Check sheet for the modelled part. Datum: model origin and axes. Units: mm. A direction names the side the tool comes from. Round coordinates to 2 decimals unless told otherwise and drop trailing zeros. Write each loop counter-clockwise with the first axis right and the second up, starting at its lowest first coordinate (ties: lowest second). Pieces come first, ordered by that corner, then holes. Notation, with made-up numbers: M 8,-17 L 54,-17 A20 cw 54,22 Z; hole C 31.5,35.25 d11. An arc over 180 degrees is marked long. Put each result on its own line as item: value.
```python
from build123d import *

# Parameters (mm, degrees)
SKETCH_1_W          = 388
SKETCH_1_H          = 260
EXTRUDE_1_DEPTH     = 50
CUT_EXTRUDE_1_DEPTH = 100
FILLET_1_R          = 10


with BuildPart() as part:
    # 草图1 → 凸台-拉伸1 (new, symmetric)
    with BuildSketch(Plane(origin=(0, 0, 0), x_dir=(0, 0, -1), z_dir=(1, 0, 0))):
        Rectangle(SKETCH_1_W, SKETCH_1_H)
    extrude(amount=EXTRUDE_1_DEPTH, both=True)

    # 草图2 → 切除-拉伸1 (cut)
    with BuildSketch(Plane(origin=(50, 0, 0), x_dir=(0, 0, -1), z_dir=(1, 0, 0))):
        with BuildLine():
            Line((-184.8, 83.5), (-180.8, 83.5))
            ThreePointArc((-180.8, 83.5), (-176.3, 79), (-180.8, 74.5))
            Line((-180.8, 74.5), (-184.8, 74.5))
            ThreePointArc((-184.8, 74.5), (-189.3, 79), (-184.8, 83.5))
        make_face()
        with BuildLine():
            Line((180.8, 83.5), (184.8, 83.5))
            ThreePointArc((184.8, 83.5), (189.3, 79), (184.8, 74.5))
            Line((184.8, 74.5), (180.8, 74.5))
            ThreePointArc((180.8, 74.5), (176.3, 79), (180.8, 83.5))
        make_face()
        with BuildLine():
            Line((180.8, -74.5), (184.8, -74.5))
            ThreePointArc((184.8, -74.5), (189.3, -79), (184.8, -83.5))
            Line((184.8, -83.5), (180.8, -83.5))
            ThreePointArc((180.8, -83.5), (176.3, -79), (180.8, -74.5))
        make_face()
        with BuildLine():
            Line((-184.8, -74.5), (-180.8, -74.5))
            ThreePointArc((-180.8, -74.5), (-176.3, -79), (-180.8, -83.5))
            Line((-180.8, -83.5), (-184.8, -83.5))
            ThreePointArc((-184.8, -83.5), (-189.3, -79), (-184.8, -74.5))
        make_face()
    extrude(amount=-CUT_EXTRUDE_1_DEPTH, mode=Mode.SUBTRACT)

    # 圆角1
    fillet_1_edges = [part.edges().sort_by_distance(p)[0] for p in [
        (0, 130, 194),
        (0, 130, -194),
        (0, -130, -194),
        (0, -130, 194),
    ]]
    fillet(fillet_1_edges, radius=FILLET_1_R)


solid = part.part
```
1. Access from +Z, -Z, +X, -X, +Y, -Y to the whole of each face (thin tool, end or side, straight path). Record for faces 4 (the flat face through (-50, 2, 3)), 5 (the cylindrical face through (0.7, -78.9, -189.3)).
Computed values:
face 4: +Z, -Z, -X, +Y, -Y
face 5: +X, -X
2. Scan line: probe 1 along Z at (x, y) = (-29, -77.5). Record every from-to range of solid material in increasing order.
Computed values:
probe 1: z = -194 to -189.04, -176.56 to 176.56, 189.04 to 194
3. Cross-section at A-A (y = -79). Enter the section's corners in (x, z).
Computed values:
outline: M -50,-194 L 50,-194 L 50,-189.3 L -50,-189.3 Z; M -50,-176.3 L 50,-176.3 L 50,176.3 L -50,176.3 Z; M -50,189.3 L 50,189.3 L 50,194 L -50,194 Z
4. Release check for a two-part mould opening along Z. For faces 1 (the cylindrical face through (0.7, 78.9, 189.3)), 2 (the cylindrical face through (0.7, -126.99, 191.15)), 3 (the flat face through (50, 2, 3)) record: +Z half, -Z half, draft (parallel to the pull), parting line (faces both ways), or undercut.
Computed values:
face 1: undercut
face 2: +Z half
face 3: draft
